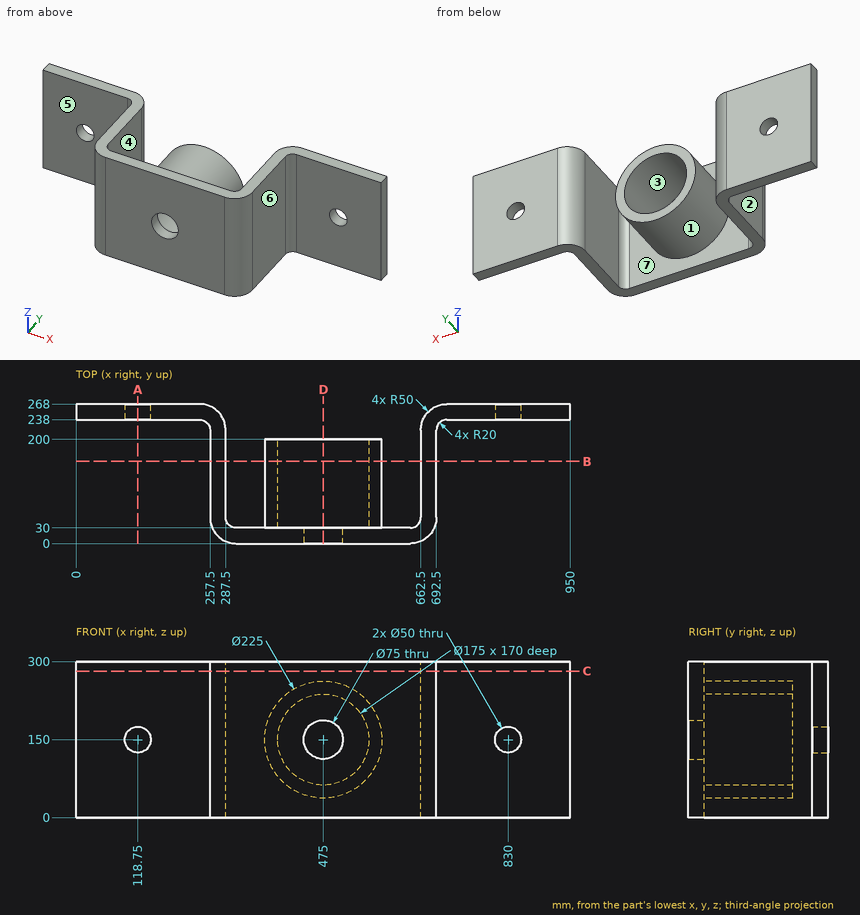
The drawing under review shows one solid part. Ordinate dimensions are in mm from its lowest x, y, z. A direction names the side the tool comes from. Round coordinates to 2 decimals unless told otherwise and drop trailing zeros. Loops run counter-clockwise (first coordinate to the right, second up) from the corner with the lowest first, then second, coordinate; pieces in that order, holes last.
Item 1: Take a section at A-A (x = 118.75). Write out the cut boundary in (y, z), then the cut area to 3 significant figures.
Determined:
outline: (238, 0) - (268, 0) - (268, 125) - (238, 125) - close; (238, 175) - (268, 175) - (268, 300) - (238, 300) - close
area: 7,500 mm2
Item 2: Take a section at D-D (x = 475). Write out the cut boundary in (y, z), then the cut area to 4 significant figures.
Determined:
outline: (0, 0) - (30, 0) - (30, 37.5) - (200, 37.5) - (200, 62.5) - (30, 62.5) - (30, 112.5) - (0, 112.5) - close; (0, 187.5) - (30, 187.5) - (30, 237.5) - (200, 237.5) - (200, 262.5) - (30, 262.5) - (30, 300) - (0, 300) - close
area: 15,250 mm2
Item 3: Take a section at B-B (y = 158). Write out the cut boundary in (x, z), then the cut area to 3 significant figures.
Determined:
outline: (257.5, 0) - (287.5, 0) - (287.5, 300) - (257.5, 300) - close; circle Ø225 at (475, 150); (662.5, 0) - (692.5, 0) - (692.5, 300) - (662.5, 300) - close; hole circle Ø175 at (475, 150)
area: 33,700 mm2
Item 4: For the marked faces 4, 5, 6 and 7, list the 3-axis set-ups (+Z, -Z, +X, -X, +Y, -Y) from which the entire face can be reached by the end or side of a thin tool; tool diameter is ignored.
Determined:
face 4: +Z, -Z, +Y
face 5: +Z, -Z, -X, -Y
face 6: +Z, -Z, +X, -Y
face 7: +Y
Item 5: For line 1 (X direction, y = 190.5, z = 146); line 2 (Z direction, x = 118.75, y = 260.5); line 3 (Z direction, x = 832.5, y = 248.5), list the stretches that pass through material, from the lowest coordinate up.
Determined:
line 1: x = 257.5 to 287.5, 362.57 to 387.59, 562.41 to 587.43, 662.5 to 692.5
line 2: z = 0 to 125, 175 to 300
line 3: z = 0 to 125.13, 174.87 to 300
Item 6: Mouldability with a two-part tool opening along Z and no side actions: class the marked faces 1, 2 and 3 as released by +Z, released by -Z, zero draft, split by the parting line, or undercut.
Determined:
face 1: split by the parting line
face 2: zero draft
face 3: undercut
Item 7: Clearance check with flat-ended pins moving along their axes: pin 1 Ø1.5 at (y, z) = (174.5, 206.5) entering from +X; pin 2 Ø12 at (x, z) = (204, 237) entering from -Y; pin 3 Ø5 at (y, z) = (188, 196) entering from -X. State where each tip first meets the part, or that it passes through.
Determined:
pin 1: stops at x = 692.5
pin 2: stops at y = 238
pin 3: stops at x = 257.5
Item 8: Take a section at C-C (z = 281.5). Write out the cut boundary in (x, y).
Determined:
outline: (0, 238) - (237.5, 238) arc R20 cw to (257.5, 218) - (257.5, 50) arc R50 ccw to (307.5, 0) - (642.5, 0) arc R50 ccw to (692.5, 50) - (692.5, 218) arc R20 cw to (712.5, 238) - (950, 238) - (950, 268) - (712.5, 268) arc R50 ccw to (662.5, 218) - (662.5, 50) arc R20 cw to (642.5, 30) - (307.5, 30) arc R20 cw to (287.5, 50) - (287.5, 218) arc R50 ccw to (237.5, 268) - (0, 268) - close
